```python
from build123d import *


with BuildPart() as part:
    # Sketch1 → Revolve1 (revolve)
    with BuildSketch(Plane.XY, mode=Mode.PRIVATE) as revolve1_sk:
        Polygon((-2.45, 29.940117832), (-2.45, -2.059882168), (-2.35, -2.059882168), (-2.35, 29.740117832), (-1.883917375, 29.740117832), (-1.883917375, 29.940117832), (-1.23, 29.940117832), (-1.23, 31.44696074), (-2.1, 31.44696074), (-2.1, 29.940117832), align=None)
    revolve(revolve1_sk.sketch.rotate(Axis((0, -5.459851486, 0), (0, 1, 0)), 270), axis=Axis((0, -5.459851486, 0), (0, 1, 0)))


solid = part.part
```
Input: part model. Units: mm. Frame: model coordinates. Coordinates: 2 decimals unless noted, no trailing zeros. Loops run counter-clockwise (first coordinate to the right, second up) from the corner with the lowest first, then second, coordinate; pieces in that order, holes last. Notation, with made-up numbers: M -1.75,71 L 56.25,71 A14 cw 56.25,80 Z; hole C 1.25,-22 d9. An arc over 180 degrees is marked long. Use a Markdown table: item, result. Add a question column.
1) Line query: L1, parallel to X at y = 30.6, z = 0; L2, parallel to X at y = 29.8, z = 0; L3, parallel to Y at x = -2, z = -0.4. Output: solid intervals per line, ascending. Write a range as from..to.
2) Section D-D, the plane z = -1.55. Return the cut outline in (x, y), plus the area to 3 significant figures.
3) Section C-C, the plane y = 20. Return the cut outline in (x, z).
4) Draft query along X for faces 1 (the flat face through (1, 31.447, 1)), 2 (the cylindrical face through (-0.631, 30.683, -2.003)), 3 (the cylindrical face through (-1.04, 30.7, -0.66)). Return one class per face: +X half, -X half, draft (parallel to the pull), parting line (faces both ways), or undercut.
5) Section A-A, the plane z = 0. Return the cut outline in (x, y), plus the area to 3 significant figures.
6) Section B-B, the plane x = 0. Return the cut outline in (y, z).
Answer below:
| question | item | result |
|---|---|---|
| 1 | L1 | -2.1..-1.23, 1.23..2.1 |
| 1 | L2 | -2.45..-1.88, 1.88..2.45 |
| 1 | L3 | 29.74..31.45 |
| 2 | outline | M -1.9,-2.06 L -1.77,-2.06 L -1.77,29.74 L -1.07,29.74 L -1.07,29.94 L 1.07,29.94 L 1.07,29.74 L 1.77,29.74 L 1.77,-2.06 L 1.9,-2.06 L 1.9,29.94 L 1.42,29.94 L 1.42,31.45 L -1.42,31.45 L -1.42,29.94 L -1.9,29.94 Z |
| 2 | area | 12.9 mm2 |
| 3 | outline | C 0,0 d4.9; hole C 0,0 d4.7 |
| 4 | face 1 | draft |
| 4 | face 2 | parting line |
| 4 | face 3 | undercut |
| 5 | outline | M -2.45,-2.06 L -2.35,-2.06 L -2.35,29.74 L -1.88,29.74 L -1.88,29.94 L -1.23,29.94 L -1.23,31.45 L -2.1,31.45 L -2.1,29.94 L -2.45,29.94 Z; M 1.23,29.94 L 1.88,29.94 L 1.88,29.74 L 2.35,29.74 L 2.35,-2.06 L 2.45,-2.06 L 2.45,29.94 L 2.1,29.94 L 2.1,31.45 L 1.23,31.45 Z |
| 5 | area | 9.21 mm2 |
| 6 | outline | M -2.06,-2.45 L 29.94,-2.45 L 29.94,-2.1 L 31.45,-2.1 L 31.45,-1.23 L 29.94,-1.23 L 29.94,-1.88 L 29.74,-1.88 L 29.74,-2.35 L -2.06,-2.35 Z; M -2.06,2.35 L 29.74,2.35 L 29.74,1.88 L 29.94,1.88 L 29.94,1.23 L 31.45,1.23 L 31.45,2.1 L 29.94,2.1 L 29.94,2.45 L -2.06,2.45 Z |
